Geometry: final body of the model. Coordinates: model frame, mm. A direction names the side the tool comes from. Give positions to 0.01 mm unless a question says otherwise; leave off trailing zeros. Loops run counter-clockwise (first coordinate to the right, second up) from the corner with the lowest first, then second, coordinate; pieces in that order, holes last. Notation, with made-up numbers: (-13.5, 80) - (2.5, 80) arc R19 ccw to (2.5, 94) - close; hole circle Ø9 at (-10.75, 5). An arc over 180 degrees is marked (long way). Answer in a Markdown table with one row per item.
from build123d import *

# Parameters (mm, degrees)
SKETCH_1_R              = 67.5
SKETCH_1_R_2            = 18
EXTRUDE_1_DEPTH         = 53
SKETCH_2_OUTSIDE_W      = 176.628
SKETCH_2_OUTSIDE_H      = 176.628
SKETCH_2_OUTSIDE_R      = 35
CUT_EXTRUDE_1_DEPTH     = 50
SKETCH_3_OUTSIDE_W      = 176.628
SKETCH_3_OUTSIDE_H      = 176.628
SKETCH_3_OUTSIDE_R      = 23
CUT_EXTRUDE_2_DEPTH     = 30
EXTRUDE_2_DEPTH         = 30
HOLE_WIZARD_M12_1_D     = 10.2
HOLE_WIZARD_M12_1_DEPTH = 5
HOLE_WIZARD_M12_1_TIP   = 3.064389157


with BuildPart() as part:
    # 草图1 → 凸台-拉伸1 (new body)
    with BuildSketch(Plane(origin=(0, 0, 0), x_dir=(1, 0, 0), z_dir=(0, 1, 0))):
        with Locations(Location((0, 0, 0), (0, 0, 270))):
            Circle(SKETCH_1_R)
        with Locations(Location((0, 0, 0), (0, 0, 270))):
            Circle(SKETCH_1_R_2, mode=Mode.SUBTRACT)
    extrude(amount=EXTRUDE_1_DEPTH)

    # 草图2 outside → 切除-拉伸1 (cut)
    with BuildSketch(Plane(origin=(0, 53, 0), x_dir=(1, 0, 0), z_dir=(0, 1, 0))):
        Rectangle(SKETCH_2_OUTSIDE_W, SKETCH_2_OUTSIDE_H)
        with Locations(Location((0, 0, 0), (0, 0, 270))):
            Circle(SKETCH_2_OUTSIDE_R, mode=Mode.SUBTRACT)
    extrude(amount=-CUT_EXTRUDE_1_DEPTH, mode=Mode.SUBTRACT)

    # 草图3 outside → 切除-拉伸2 (cut)
    with BuildSketch(Plane(origin=(0, 53, 0), x_dir=(1, 0, 0), z_dir=(0, 1, 0))):
        Rectangle(SKETCH_3_OUTSIDE_W, SKETCH_3_OUTSIDE_H)
        with Locations(Location((0, 0, 0), (0, 0, 270))):
            Circle(SKETCH_3_OUTSIDE_R, mode=Mode.SUBTRACT)
    extrude(amount=-CUT_EXTRUDE_2_DEPTH, mode=Mode.SUBTRACT)

    # 草图4 → 凸台-拉伸2 (add)
    with BuildSketch(Plane(origin=(0, 53, 0), x_dir=(1, 0, 0), z_dir=(0, 1, 0))):
        Polygon((0, 25), (4.5, 25), (4.5, 18.659112383), (-4.5, 18.659112383), (-4.5, 25), align=None)
        Polygon((10.012004382, 16.375965412), (14.495689014, 20.859650045), (17.67766953, 17.67766953), (20.859650045, 14.495689014), (16.375965412, 10.012004382), align=None)
        Polygon((18.659112383, 4.5), (25, 4.5), (25, 0), (25, -4.5), (18.659112383, -4.5), align=None)
        Polygon((16.375965412, -10.012004382), (20.859650045, -14.495689014), (17.67766953, -17.67766953), (14.495689014, -20.859650045), (10.012004382, -16.375965412), align=None)
        Polygon((4.5, -18.659112383), (4.5, -25), (0, -25), (-4.5, -25), (-4.5, -18.659112383), align=None)
        Polygon((-10.012004382, -16.375965412), (-14.495689014, -20.859650045), (-17.67766953, -17.67766953), (-20.859650045, -14.495689014), (-16.375965412, -10.012004382), align=None)
        Polygon((-18.659112383, -4.5), (-25, -4.5), (-25, 0), (-25, 4.5), (-18.659112383, 4.5), align=None)
        Polygon((-16.375965412, 10.012004382), (-20.859650045, 14.495689014), (-17.67766953, 17.67766953), (-14.495689014, 20.859650045), (-10.012004382, 16.375965412), align=None)
    extrude(amount=-EXTRUDE_2_DEPTH)

    # M12 螺纹孔的螺纹孔钻头1
    with Locations(Plane(origin=(0, 3, 0), x_dir=(1, 0, 0), z_dir=(0, 1, 0))):
        with Locations((0, 55), (-47.631397208, 27.5), (-47.631397208, -27.5), (0, -55), (47.631397208, -27.5), (47.631397208, 27.5)):
            Hole(HOLE_WIZARD_M12_1_D / 2, depth=HOLE_WIZARD_M12_1_DEPTH)
            with Locations((0, 0, -(HOLE_WIZARD_M12_1_DEPTH + HOLE_WIZARD_M12_1_TIP / 2))):  # 118° drill point
                Cone(0, HOLE_WIZARD_M12_1_D / 2, HOLE_WIZARD_M12_1_TIP, mode=Mode.SUBTRACT)


solid = part.part
Q1. Reachability of faces 4 (the cylindrical face through (-21, 13, -28)), 5 (the cylindrical face through (-21.225, 38.21, -8.86)), 6 (the flat face through (-25, 38, 0)), 7 (the cylindrical face through (-8.86, 38.21, 21.225)) from +Z, -Z, +X, -X, +Y, -Y: full face, straight path, thin tool, end or side. Return the list, or none.
Check values:
| item | result |
|---|---|
| face 4 | +Y |
| face 5 | -X, +Y |
| face 6 | +Z, -Z, -X, +Y |
| face 7 | +Z, +Y |
Q2. Material intervals for line 1 along X through (y, z) = (2.1, 27.5); line 2 along X through (y, z) = (48, -19.5); line 3 along Y through (x, z) = (-21.5, -35), sorted ascending.
Check values:
| item | result |
|---|---|
| line 1 | -61.64 to -52.73, -42.53 to 42.53, 52.73 to 61.64 |
| line 2 | -15.86 to -13.14, -12.2 to 12.2, 13.14 to 15.86 |
| line 3 | 0 to 3 |
Q3. Draft query along Z for faces 1 (the flat face through (0, 38, 25)), 2 (the cylindrical face through (21.225, 38.21, 8.86)), 3 (the flat face through (0, 38, -25)). Return one class per face: pulls with the +Z half, pulls with the -Z half, needs draft (parallel to the pull), parting line crosses it, or undercut.
Check values:
| item | result |
|---|---|
| face 1 | pulls with the +Z half |
| face 2 | undercut |
| face 3 | pulls with the -Z half |
Q4. Cut plane C-C (x = 48.5). Output: boundary loops of the cut face in (y, z), and give its area (3 significant figures).
Check values:
| item | result |
|---|---|
| outline | (0, -46.95) - (3, -46.95) - (3, -32.53) - (0, -32.53) - close; (0, -22.47) - (3, -22.47) - (3, 22.47) - (0, 22.47) - close; (0, 32.53) - (3, 32.53) - (3, 46.95) - (0, 46.95) - close |
| area | 221 mm² |
Q5. Cut plane D-D (z = 27.5). Output: boundary loops of the cut face in (x, y).
Check values:
| item | result |
|---|---|
| outline | (-61.64, 0) - (-52.73, 0) - (-52.73, 3) - (-61.64, 3) - close; (-42.53, 0) - (42.53, 0) - (42.53, 3) - (21.65, 3) - (21.65, 23) - (-21.65, 23) - (-21.65, 3) - (-42.53, 3) - close; (52.73, 0) - (61.64, 0) - (61.64, 3) - (52.73, 3) - close |
Q6. Cut plane B-B (z = 0). Output: boundary loops of the cut face in (x, y), and give its area (3 significant figures).
Check values:
| item | result |
|---|---|
| outline | (-67.5, 0) - (-18, 0) - (-18, 53) - (-25, 53) - (-25, 23) - (-35, 23) - (-35, 3) - (-67.5, 3) - close; (18, 0) - (67.5, 0) - (67.5, 3) - (35, 3) - (35, 23) - (25, 23) - (25, 53) - (18, 53) - close |
| area | 1,400 mm² |
Q7. First-contact query: pin 1 (2 mm diameter, centred on y = 9, z = -9, fed in from +X); pin 2 (8 mm diameter, centred on x = -22, y = 39.5, fed in from +Z); pin 3 (0.7 mm diameter, centred on y = 36.5, z = 24, fed in from -X); pin 4 (6 mm diameter, centred on x = -47.63, z = 27.5, fed in from -Y). Flat tips, straight axial feed; report the tip coordinate or a pass-through.
Check values:
| item | result |
|---|---|
| pin 1 | x = 34.07 |
| pin 2 | z = 17.36 |
| pin 3 | x = -4.5 |
| pin 4 | through |
Q8. Cut plane A-A (x = 0). Output: boundary loops of the cut face in (y, z).
Check values:
| item | result |
|---|---|
| outline | (0, -67.5) - (3, -67.5) - (3, -60.1) - (0, -60.1) - close; (0, -49.9) - (3, -49.9) - (3, -35) - (23, -35) - (23, -25) - (53, -25) - (53, -18) - (0, -18) - close; (0, 18) - (53, 18) - (53, 25) - (23, 25) - (23, 35) - (3, 35) - (3, 49.9) - (0, 49.9) - close; (0, 60.1) - (3, 60.1) - (3, 67.5) - (0, 67.5) - close |
